from build123d import *

# Parameters (mm, degrees)
SKETCH_1_R          = 38
EXTRUDE_1_DEPTH     = 110
SKETCH_4_OUTSIDE_W  = 126.97
SKETCH_4_OUTSIDE_H  = 126.97
SKETCH_4_OUTSIDE_R  = 31.5
CUT_EXTRUDE_1_DEPTH = 21
SKETCH_5_OUTSIDE_W  = 126.97
SKETCH_5_OUTSIDE_H  = 126.97
SKETCH_5_OUTSIDE_R  = 31.5
CUT_EXTRUDE_2_DEPTH = 21
FILLET_1_R          = 5
SKETCH_2_R          = 5.478928785
SKETCH_2_R_2        = 5.511284945
EXTRUDE_2_DEPTH     = 2


with BuildPart() as part:
    # 草图1 → 凸台-拉伸1 (new, symmetric)
    with BuildSketch(Plane.XY):
        Circle(SKETCH_1_R)
    extrude(amount=EXTRUDE_1_DEPTH, both=True)

    # 草图4 outside → 切除-拉伸1 (cut)
    with BuildSketch(Plane.XY.offset(110)):
        Rectangle(SKETCH_4_OUTSIDE_W, SKETCH_4_OUTSIDE_H)
        Circle(SKETCH_4_OUTSIDE_R, mode=Mode.SUBTRACT)
    extrude(amount=-CUT_EXTRUDE_1_DEPTH, mode=Mode.SUBTRACT)

    # 草图5 outside → 切除-拉伸2 (cut)
    with BuildSketch(Plane(origin=(0, 0, -110), x_dir=(-1, 0, 0), z_dir=(0, 0, -1))):
        Rectangle(SKETCH_5_OUTSIDE_W, SKETCH_5_OUTSIDE_H)
        with Locations(Location((0, 0, 0), (0, 0, 180))):
            Circle(SKETCH_5_OUTSIDE_R, mode=Mode.SUBTRACT)
    extrude(amount=-CUT_EXTRUDE_2_DEPTH, mode=Mode.SUBTRACT)

    # 圆角1
    fillet_1_edges = [part.edges().sort_by_distance(p)[0] for p in [
        (-31.5, 0, 110),
        (-38, 0, -89),
        (-31.5, 0, -110),
        (-38, 0, 89),
    ]]
    fillet(fillet_1_edges, radius=FILLET_1_R)

    # 草图2 → 凸台-拉伸2 (add)
    with BuildSketch(Plane(origin=(0, 0, -110), x_dir=(-1, 0, 0), z_dir=(0, 0, -1))):
        with Locations(Location((0, 15.014240139, 0), (0, 0, 180))):
            Circle(SKETCH_2_R)
        with Locations(Location((0, -16.315898799, 0), (0, 0, 180))):
            Circle(SKETCH_2_R_2)
    extrude(amount=EXTRUDE_2_DEPTH)


solid = part.part
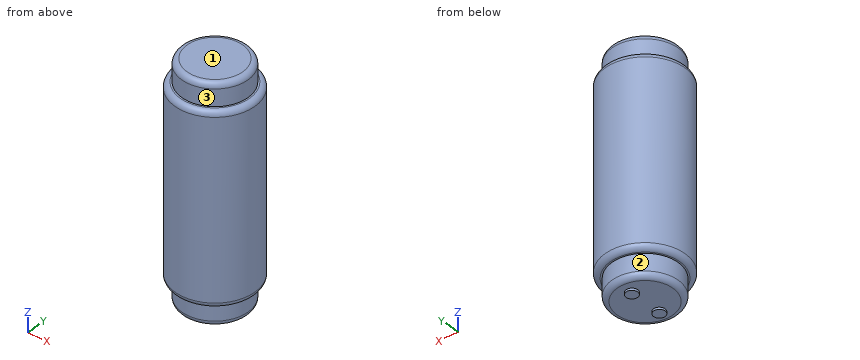
Design review of the part built by this model. Coordinates are the model's own, in mm. Face numbers are marked on the shaded views. A direction names the side the tool comes from. Coordinates: 2 decimals unless noted, no trailing zeros. Loops run counter-clockwise (first coordinate to the right, second up) from the corner with the lowest first, then second, coordinate; pieces in that order, holes last. Notation, with made-up numbers: M 9.5,30 L 64.5,30 A15 cw 64.5,36 Z; hole C -12,20.25 d2. An arc over 180 degrees is marked long. Use one line per item in the form item = value.
(1) For the marked faces 1, 2 and 3, list the 3-axis set-ups (+Z, -Z, +X, -X, +Y, -Y) from which the entire face can be reached by the end or side of a thin tool; tool diameter is ignored.
Return value:
face_1 = +Z, +X, -X, +Y, -Y
face_2 = -Z
face_3 = +Z
(2) Clearance check with flat-ended pins moving along their axes: P1, Ø8, axis at y = -26.5, z = 73.5, coming from the +X side; P2, Ø10, axis at y = -19.5, z = -75, coming from the +X side; P3, Ø10, axis at y = 7.5, z = 73, coming from the +X side. State where each tip first meets the part, or that it passes through.
Return value:
P1 = 30.62
P2 = 35.12
P3 = 37.92
(3) For line 1 along Y through (x, z) = (-17, -99); line 2 along Z through (x, y) = (-15, -10); line 3 along X through (y, z) = (-0.5, -19.5), list the stretches that pass through material, from the lowest coordinate up. Write a range as from..to.
Return value:
line_1 = -26.52..26.52
line_2 = -110..110
line_3 = -38..38
(4) Consider section B-B (y = 0). Write out the cut boundary in (x, z), and give its area (3 significant figures).
Return value:
outline = M -38,-84 A5 ccw -33,-89 L -31.5,-89 L -31.5,-105 A5 ccw -26.5,-110 L 26.5,-110 A5 ccw 31.5,-105 L 31.5,-89 L 33,-89 A5 ccw 38,-84 L 38,84 A5 ccw 33,89 L 31.5,89 L 31.5,105 A5 ccw 26.5,110 L -26.5,110 A5 ccw -31.5,105 L -31.5,89 L -33,89 A5 ccw -38,84 Z
area = 16,100 mm2
(5) Consider section A-A (x = 0). Write out the cut boundary in (y, z), and give its area (3 significant figures).
Return value:
outline = M -38,-84 A5 ccw -33,-89 L -31.5,-89 L -31.5,-105 A5 ccw -26.5,-110 L -21.83,-110 L -21.83,-112 L -10.8,-112 L -10.8,-110 L 9.54,-110 L 9.54,-112 L 20.49,-112 L 20.49,-110 L 26.5,-110 A5 ccw 31.5,-105 L 31.5,-89 L 33,-89 A5 ccw 38,-84 L 38,84 A5 ccw 33,89 L 31.5,89 L 31.5,105 A5 ccw 26.5,110 L -26.5,110 A5 ccw -31.5,105 L -31.5,89 L -33,89 A5 ccw -38,84 Z
area = 16,200 mm2
(6) Consider section C-C (z = 82). Write out the cut boundary in (x, y).
Return value:
outline = C 0,0 d76
